Design review of the part built by this model. Coordinates are the model's own, in mm. A direction names the side the tool comes from. Give positions to 0.01 mm unless a question says otherwise; leave off trailing zeros. Order: outer loops, then holes, each group sorted by start corner. A loop starts at its lowest first (then second) coordinate and runs counter-clockwise, first axis right, second up. Notation, with made-up numbers: (1.25, -34.75) -> (48.25, -34.75) arc R18 ccw to (48.25, -6.75) -> close; hole circle Ø11 at (89.25, 85). An arc over 180 degrees is marked (long way). One line per item, written item: value. Start each with the question number.
1) For pin 1 (4 mm diameter, centred on y = 0, z = 36.5, fed in from +X); pin 2 (2.5 mm diameter, centred on x = 0, y = 0, fed in from +Z); pin 3 (1.5 mm diameter, centred on x = 1, z = -8, fed in from +Y), all flat-tipped, find the tip position at first contact; note any pin that passes through.
2) The part is to be moulded in two halves that separate along Y. For faces 4 (the face through (0, -7.931, 1)), 5 (the face through (-10, 7, 1)), 6 (the face through (7.931, 0, 1)), 7 (the face through (-7, 10, 1)), say which applies: released by +Y, released by -Y, zero draft, split by the parting line, or undercut.
3) Consider section C-C (z = -42). State the section outline as (x, y) points.
4) Consider section A-A (x = 0). State the section outline as (y, z) points.
5) Tool access review of faces 1 (the face through (0, 7.931, 1)), 2 (the face through (-7.931, 0, 1)), 3 (the face through (-10, -7, 1)): name each direction out of +Z, -Z, +X, -X, +Y, -Y from which nothing blocks a thin tool from reaching the whole face with its end or side.
6) Wall thickness on line 1 along Y through (x, z) = (0, 45.5); line 2 along X through (y, z) = (2, 62.5); line 3 along X through (y, z) = (8.25, 63.5): over which ranges is each line inside the solid? List them lowest first. Write a range as from..to.
from build123d import *

# Parameters (mm, degrees)
SKETCH_1_W               = 20
SKETCH_1_H               = 20
SKETCH_1_R               = 1.94442565
EXTRUDE_1_DEPTH          = 90
CUT_EXTRUDE_1_DEPTH      = 181.554700853
PATTERN_CIRCULAR_1_COUNT = 4


with BuildPart() as part:
    # 草图1 → 凸台-拉伸1 (new, symmetric)
    with BuildSketch(Plane.XY):
        Rectangle(SKETCH_1_W, SKETCH_1_H)
        with Locations(Location((0, 0, 0), (0, 0, 180))):
            Circle(SKETCH_1_R, mode=Mode.SUBTRACT)
    extrude(amount=EXTRUDE_1_DEPTH, both=True)

    # 草图2 → 切除-拉伸1 (cut, symmetric)
    with BuildSketch(Plane.XY.offset(90)):
        Polygon((-32.933615203, 60.643738676), (-3.694439046, 10), (-2.5, 7.931170886), (2.5, 7.931170886), (3.694439046, 10), (32.933615203, 60.643738676), (32.933615203, 177.600443305), (-32.933615203, 177.600443305), align=None)
    cut_extrude_1 = extrude(amount=CUT_EXTRUDE_1_DEPTH, both=True, mode=Mode.SUBTRACT)

    # 阵列(圆周)1: 切除-拉伸1 ×4 about axis
    pattern_circular_1_axis = Axis((0, 0, 90), (0, 0, -1))
    for i in range(1, PATTERN_CIRCULAR_1_COUNT):
        add(cut_extrude_1.rotate(pattern_circular_1_axis, i * 360 / PATTERN_CIRCULAR_1_COUNT), mode=Mode.SUBTRACT)


solid = part.part
Checked values:
1. pin 1: stops at x = 7.93
1. pin 2: passes through
1. pin 3: stops at y = 7.93
2. face 4: released by -Y
2. face 5: zero draft
2. face 6: undercut
2. face 7: released by +Y
3. outline: (-10, -10) -> (-3.69, -10) -> (-2.5, -7.93) -> (2.5, -7.93) -> (3.69, -10) -> (10, -10) -> (10, -3.69) -> (7.93, -2.5) -> (7.93, 2.5) -> (10, 3.69) -> (10, 10) -> (3.69, 10) -> (2.5, 7.93) -> (-2.5, 7.93) -> (-3.69, 10) -> (-10, 10) -> (-10, 3.69) -> (-7.93, 2.5) -> (-7.93, -2.5) -> (-10, -3.69) -> close; hole circle Ø3.89 at (0, 0)
4. outline: (-7.93, -90) -> (-1.94, -90) -> (-1.94, 90) -> (-7.93, 90) -> close; (1.94, -90) -> (7.93, -90) -> (7.93, 90) -> (1.94, 90) -> close
5. face 1: +Z, -Z, +Y
5. face 2: +Z, -Z, -X
5. face 3: +Z, -Z, -X, +Y, -Y
6. line 1: y = -7.93..-1.94, 1.94..7.93
6. line 2: x = -7.93..7.93
6. line 3: x = -10..-2.68, 2.68..10
